from build123d import *

# Parameters (mm, degrees)
SKETCH1_W           = 70
SKETCH1_H           = 55
SKETCH1_W_2         = 40
SKETCH1_H_2         = 40
BOSS_EXTRUDE1_DEPTH = 30
SKETCH2_W           = 70
SKETCH2_H           = 20
BOSS_EXTRUDE2_DEPTH = 30
SKETCH3_R           = 8
CUT_EXTRUDE1_DEPTH  = 30
SKETCH4_R           = 17.338439929
SKETCH4_R_2         = 8
BOSS_EXTRUDE3_DEPTH = 30
SKETCH5_R           = 5
CUT_EXTRUDE2_DEPTH  = 6
SKETCH6_R           = 4.5
BOSS_EXTRUDE4_DEPTH = 5


with BuildPart() as part:
    # Sketch1 → Boss-Extrude1 (new body)
    with BuildSketch(Plane(origin=(0, 0, 0), x_dir=(1, 0, 0), z_dir=(0, 1, 0))):
        Rectangle(SKETCH1_W, SKETCH1_H)
        Rectangle(SKETCH1_W_2, SKETCH1_H_2, mode=Mode.SUBTRACT)
    extrude(amount=BOSS_EXTRUDE1_DEPTH)

    # Sketch2 → Boss-Extrude2 (add)
    with BuildSketch(Plane(origin=(0, 30, 0), x_dir=(1, 0, 0), z_dir=(0, 1, 0))):
        with Locations((0, 37.5)):
            Rectangle(SKETCH2_W, SKETCH2_H)
    extrude(amount=-BOSS_EXTRUDE2_DEPTH)

    # Sketch3 → Cut-Extrude1 (cut)
    with BuildSketch(Plane.XZ):
        with Locations((0, -42)):
            Circle(SKETCH3_R)
    extrude(amount=-CUT_EXTRUDE1_DEPTH, mode=Mode.SUBTRACT)

    # Sketch4 → Boss-Extrude3 (add)
    with BuildSketch(Plane.XZ):
        with Locations((0, -42)):
            Circle(SKETCH4_R)
        with Locations(Location((0, -42, 0), (0, 0, 270))):
            Circle(SKETCH4_R_2, mode=Mode.SUBTRACT)
    extrude(amount=-BOSS_EXTRUDE3_DEPTH)

    # Sketch5 → Cut-Extrude2 (cut)
    with BuildSketch(Plane.ZY.offset(35)):
        with Locations((12.5, 15)):
            Circle(SKETCH5_R)
        with Locations((-12.5, 15)):
            Circle(SKETCH5_R)
    cut_extrude2 = extrude(amount=-CUT_EXTRUDE2_DEPTH, mode=Mode.SUBTRACT)

    # Sketch6 → Boss-Extrude4 (add)
    # profile 1 of 2: a face of its own
    with BuildSketch(Plane.ZY.offset(29)):
        with Locations((-12.5, 15)):
            Circle(SKETCH6_R)
        Polygon((-10.422763648, 13.355760931), (-10.03742902, 15.976819916), (-12.114665372, 17.621058985), (-14.577236352, 16.644239069), (-14.96257098, 14.023180084), (-12.885334628, 12.378941015), align=None, mode=Mode.SUBTRACT)
    # profile 2 of 2: a face of its own
    with BuildSketch(Plane.ZY.offset(29)):
        with Locations((12.5, 15)):
            Circle(SKETCH6_R)
        Polygon((14.569670203, 13.355760931), (14.958787905, 15.970267439), (12.889117702, 17.614506508), (10.430329797, 16.644239069), (10.041212095, 14.029732561), (12.110882298, 12.385493492), align=None, mode=Mode.SUBTRACT)
    boss_extrude4 = extrude(amount=BOSS_EXTRUDE4_DEPTH)

    # Mirror1: Cut-Extrude2, Boss-Extrude4 across plane
    add(cut_extrude2.mirror(Plane(origin=(0, 0, 0), x_dir=(0, 0, 1), z_dir=(1, 0, 0))), mode=Mode.SUBTRACT)
    add(boss_extrude4.mirror(Plane(origin=(0, 0, 0), x_dir=(0, 0, 1), z_dir=(1, 0, 0))))


solid = part.part
CAD build for the part. Positions are in the model's coordinates, mm. A direction names the side the tool comes from. Coordinates: 2 decimals unless noted, no trailing zeros. Order: outer loops, then holes, each group sorted by start corner. A loop starts at its lowest first (then second) coordinate and runs counter-clockwise, first axis right, second up. Notation, with made-up numbers: (-32, -31) -> (27, -31) arc R32 cw to (27, 1) -> close; hole circle Ø1 at (-24.5, -20). An arc over 180 degrees is marked (long way). Answer in a Markdown table with one row per item.
1) Band-saw the part on A-A (z = 5). List the corners of the cut face in (x, y), and give its area (3 significant figures).
Check values:
| item | result |
|---|---|
| outline | (-35, 0) -> (-20, 0) -> (-20, 30) -> (-35, 30) -> close; (20, 0) -> (35, 0) -> (35, 30) -> (20, 30) -> close |
| area | 900 mm2 |
2) Flat gauge pins, fed straight in: P1, Ø5.5, axis at y = 16, z = -11.5, coming from the +X side; P2, Ø2.5, axis at y = 15.5, z = -11.5, coming from the -X side; P3, Ø14.5, axis at x = 0, z = -42, coming from the +Y side; P4, Ø6, axis at x = -8, y = 21, coming from the -Z side. Where does each tip first touch, or does it go through?
Check values:
| item | result |
|---|---|
| P1 | x = 34 |
| P2 | x = -29 |
| P3 | through |
| P4 | z = -58.6 |
3) Band-saw the part on B-B (x = 9). List the corners of the cut face in (y, z).
Check values:
| item | result |
|---|---|
| outline | (0, -56.82) -> (30, -56.82) -> (30, -20) -> (0, -20) -> close; (0, 20) -> (30, 20) -> (30, 27.5) -> (0, 27.5) -> close |
4) Band-saw the part on C-C (y = 22). List the corners of the cut face in (x, z), and give its area (3 significant figures).
Check values:
| item | result |
|---|---|
| outline | (-35, -47.5) -> (-16.44, -47.5) arc R17.34 ccw to (16.44, -47.5) -> (35, -47.5) -> (35, 27.5) -> (-35, 27.5) -> close; hole (-20, -20) -> (20, -20) -> (20, 20) -> (-20, 20) -> close; hole circle Ø16 at (0, -42) |
| area | 3,730 mm2 |
5) Mould opens along Y. For faces 1 (the face through (-31.465, 16.787, -11.062)), 2 (the face through (0, 15, 20)) say: pulls with the +Y half, pulls with the -Y half, needs draft (parallel to the pull), parting line crosses it, or undercut.
Check values:
| item | result |
|---|---|
| face 1 | undercut |
| face 2 | needs draft |
6) Band-saw the part on D-D (x = 25). List the corners of the cut face in (y, z), and give its area (3 significant figures).
Check values:
| item | result |
|---|---|
| outline | (0, -47.5) -> (30, -47.5) -> (30, 27.5) -> (0, 27.5) -> close |
| area | 2,250 mm2 |
7) Drill centre lines: line 1 (X direction, y = 11.75, z = -9); line 2 (X direction, y = 27.75, z = -12); line 3 (Z direction, x = -4, y = 5.75). Where is each one in solid material? Low to high.
Check values:
| item | result |
|---|---|
| line 1 | -29 to -20, 20 to 29 |
| line 2 | -35 to -20, 20 to 35 |
| line 3 | -58.87 to -48.93, -35.07 to -20, 20 to 27.5 |
8) Which spindle directions (+Z, -Z, +X, -X, +Y, -Y) get a long thin tool onto all of the face, cutting with end or side? Do faces 3 (the face through (-31.465, 12.864, 13.323)), 4 (the face through (20, 15, 0)), 5 (the face through (31.465, 14.648, -10.233)). Say none if no direction does.
Check values:
| item | result |
|---|---|
| face 3 | -X |
| face 4 | +Y, -Y |
| face 5 | +X |
